Check sheet for the modelled part. Datum: model origin and axes. Units: mm. Face numbers are marked on the shaded views. Round coordinates to 2 decimals unless told otherwise and drop trailing zeros. Loops run counter-clockwise (first coordinate to the right, second up) from the corner with the lowest first, then second, coordinate; pieces in that order, holes last. Notation, with made-up numbers: (-28, 68) -> (-10, 68) arc R24 ccw to (-10, 91) -> close; hole circle Ø11 at (1.5, -30). An arc over 180 degrees is marked (long way). One line per question, with ' | ' between items.
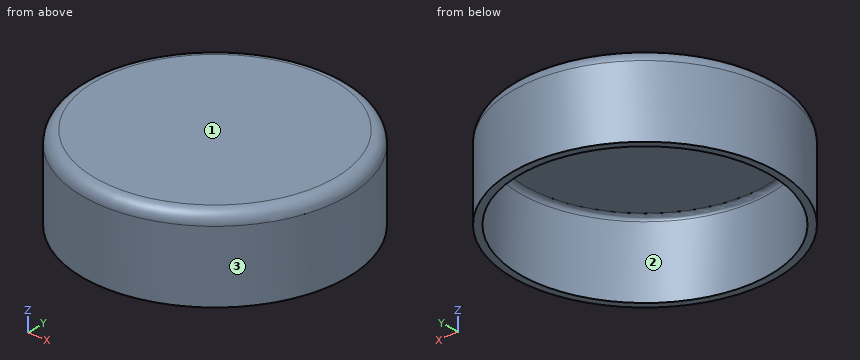
```python
from build123d import *

# Parameters (mm, degrees)
SKETCH1_R           = 109.5
BOSS_EXTRUDE1_DEPTH = 69
SHELL1_T            = -6
FILLET1_R           = 10
FILLET2_R           = 4


with BuildPart() as part:
    # Sketch1 → Boss-Extrude1 (new body)
    with BuildSketch(Plane.XY):
        Circle(SKETCH1_R)
    extrude(amount=BOSS_EXTRUDE1_DEPTH)

    # Shell1
    shell1_openings = [part.faces().sort_by_distance(p)[0] for p in [
        (0, 0, 0),
    ]]
    offset(amount=SHELL1_T, openings=shell1_openings, kind=Kind.INTERSECTION)

    # Fillet1
    fillet1_edges = [part.edges().sort_by_distance(p)[0] for p in [
        (-109.5, 0, 69),
    ]]
    fillet(fillet1_edges, radius=FILLET1_R)

    # Fillet2
    fillet2_edges = [part.edges().sort_by_distance(p)[0] for p in [
        (-103.5, 0, 63),
    ]]
    fillet(fillet2_edges, radius=FILLET2_R)


solid = part.part
```
(1) Scan lines: probe 1 along Y at (x, z) = (0, 44.5); probe 2 along Z at (x, y) = (-3, -57); probe 3 along Y at (x, z) = (58.5, 7.5). Record each from-to range of solid material in increasing order.
Answer:
probe 1: y = -109.5 to -103.5, 103.5 to 109.5 | probe 2: z = 63 to 69 | probe 3: y = -92.56 to -85.38, 85.38 to 92.56
(2) Sectioned sample at B-B, the plane z = 7. Record the cut outline in (x, y).
Answer:
outline: circle Ø219 at (0, 0); hole circle Ø207 at (0, 0)
(3) Mould release check, pull along Y, two halves, no side actions. Record for the marked faces 1, 2 and 3: +Y half, -Y half, draft (parallel to the pull), parting line (faces both ways), or undercut.
Answer:
face 1: draft | face 2: undercut | face 3: parting line
(4) Go/stop test with flat-tipped pins: pin 1 (1 mm diameter, centred on y = -42.5, z = 30, fed in from +X); pin 2 (10 mm diameter, centred on x = 67, z = 27, fed in from +Y); pin 3 (1 mm diameter, centred on x = 67.5, z = 60.5, fed in from +Y). Record where each tip stops, or that it passes through.
Answer:
pin 1: stops at x = 101.12 | pin 2: stops at y = 90.26 | pin 3: stops at y = 86.48
(5) Sectioned sample at A-A, the plane x = 0. Record the cut outline in (y, z), and give its area (3 significant figures).
Answer:
outline: (-109.5, 0) -> (-103.5, 0) -> (-103.5, 59) arc R4 cw to (-99.5, 63) -> (99.5, 63) arc R4 cw to (103.5, 59) -> (103.5, 0) -> (109.5, 0) -> (109.5, 59) arc R10 ccw to (99.5, 69) -> (-99.5, 69) arc R10 ccw to (-109.5, 59) -> close | area: 2,030 mm2
